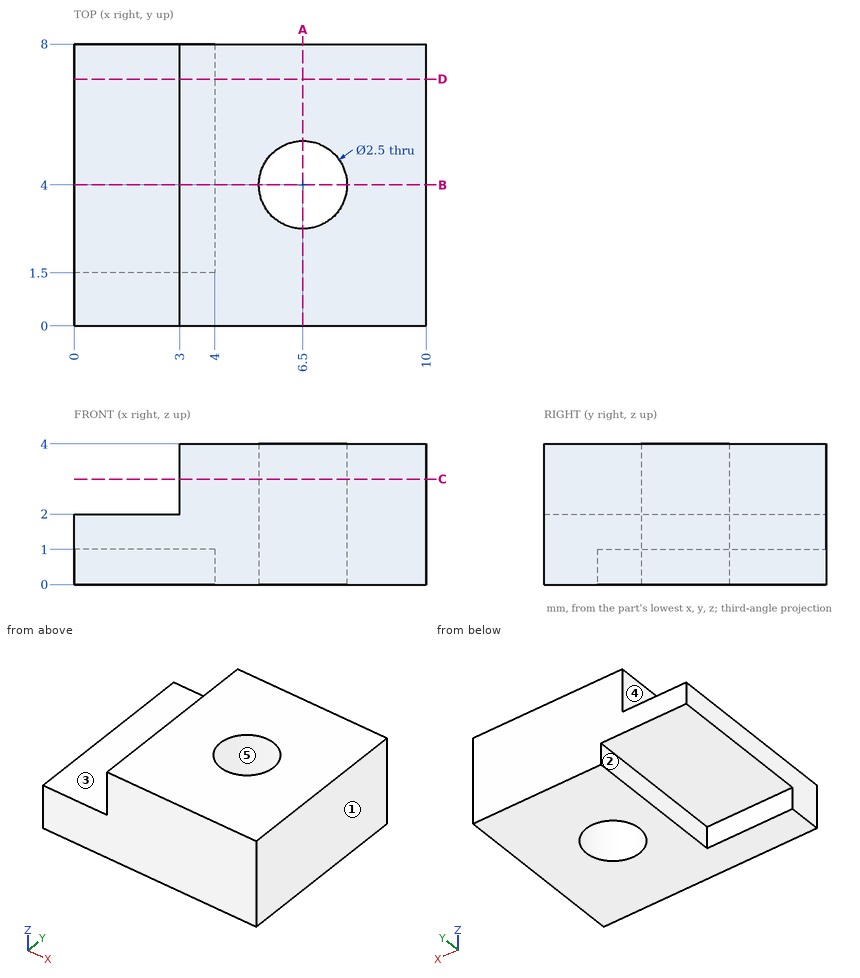
Source: three-view drawing plus pictorial views. Frame: mm from the lowest corner of the part. A direction names the side the tool comes from. Give positions to 0.01 mm unless a question says otherwise; leave off trailing zeros. Order: outer loops, then holes, each group sorted by start corner. A loop starts at its lowest first (then second) coordinate and runs counter-clockwise, first axis right, second up. Notation, with made-up numbers: (-11.75, 56.5) - (35.25, 56.5) arc R15 cw to (35.25, 70.5) - close; hole circle Ø11 at (51, -11). An arc over 180 degrees is marked (long way). Answer as a JSON object with one key per item and string values. Group by question number.
Q1. Line query: probe 1 along Y at (x, z) = (6.5, 2.6); probe 2 along X at (y, z) = (1.5, 2.35); probe 3 along X at (y, z) = (2.5, 0.75). Output: solid intervals per line, ascending.
Q2. First-contact query: pin 1 Ø0.5 at (x, z) = (2.5, 0.5) entering from +Y; pin 2 Ø2 at (x, y) = (1.5, 5.5) entering from -Z; pin 3 Ø2 at (y, z) = (3, 3.5) entering from -X. Flat tips, straight axial feed; report the tip coordinate or a pass-through.
Q3. Cut plane D-D, the plane y = 7. Output: boundary loops of the cut face in (x, z), then the cut area to 3 significant figures.
Q4. Set-up query: the marked faces 1 and 2. Return all of +Z, -Z, +X, -X, +Y, -Y with unobstructed straight access to the full face (end or side cutting, diameter ignored); none if empty.
Q5. Cut plane C-C, the plane z = 3. Output: boundary loops of the cut face in (x, y).
Q6. Mould query, pull axis X, two halves, no side actions, for the marked faces 3, 4 and 5. Classes: pulls with the +X half, pulls with the -X half, needs draft (parallel to the pull), parting line crosses it, or undercut.
Q7. Cut plane A-A, the plane x = 6.5. Output: boundary loops of the cut face in (y, z).
Q8. Cut plane B-B, the plane y = 4. Output: boundary loops of the cut face in (x, z), then the cut area to 3 significant figures.
Results:
{
 "1": {"probe 1": "0 to 2.75, 5.25 to 8", "probe 2": "3 to 10", "probe 3": "4 to 10"},
 "2": {"pin 1": "y = 1.5", "pin 2": "z = 1", "pin 3": "x = 3"},
 "3": {"outline": "(0, 1) - (4, 1) - (4, 0) - (10, 0) - (10, 4) - (3, 4) - (3, 2) - (0, 2) - close", "area": "30.0 mm^2"},
 "4": {"face 1": "+Z, -Z, +X, +Y, -Y", "face 2": "-Z, -X, +Y"},
 "5": {"outline": "(3, 0) - (10, 0) - (10, 8) - (3, 8) - close; hole circle Ø2.5 at (6.5, 4)"},
 "6": {"face 3": "needs draft", "face 4": "pulls with the -X half", "face 5": "undercut"},
 "7": {"outline": "(0, 0) - (2.75, 0) - (2.75, 4) - (0, 4) - close; (5.25, 0) - (8, 0) - (8, 4) - (5.25, 4) - close"},
 "8": {"outline": "(0, 1) - (4, 1) - (4, 0) - (5.25, 0) - (5.25, 4) - (3, 4) - (3, 2) - (0, 2) - close; (7.75, 0) - (10, 0) - (10, 4) - (7.75, 4) - close", "area": "20.0 mm^2"}
}
